from build123d import *

# Parameters (mm, degrees)
SKETCH1_W                = 15
SKETCH1_H                = 15
BOSS_EXTRUDE1_DEPTH      = 730
SKETCH2_R                = 5
BOSS_EXTRUDE2_DEPTH      = 8
SKETCH4_W                = 15
SKETCH4_H                = 15
BOSS_EXTRUDE3_DEPTH      = 198
SKETCH5_W                = 15
SKETCH5_H                = 730
BOSS_EXTRUDE4_DEPTH      = 15
BOSS_EXTRUDE5_START      = 8
SKETCH6_R                = 5
BOSS_EXTRUDE5_DEPTH      = 8
FILLET1_R                = 6
BOSS_EXTRUDE6_DEPTH      = 20
BOSS_EXTRUDE6_DEPTH_BACK = 250
SKETCH7_R                = 5


with BuildPart() as part:
    # Sketch1 → Boss-Extrude1 (new body)
    with BuildSketch(Plane(origin=(0, 0, 0), x_dir=(1, 0, 0), z_dir=(0, 1, 0))):
        Rectangle(SKETCH1_W, SKETCH1_H)
    extrude(amount=BOSS_EXTRUDE1_DEPTH)

    # Sketch2 → Boss-Extrude2 (add)
    with BuildSketch(Plane(origin=(0, 0, -7.5), x_dir=(-1, 0, 0), z_dir=(0, 0, -1))):
        with Locations(Location((0, 10, 0), (0, 0, 180))):
            Circle(SKETCH2_R)
    extrude(amount=BOSS_EXTRUDE2_DEPTH)

    # Sketch4 → Boss-Extrude3 (add)
    with BuildSketch(Plane.XY.offset(7.5)):
        with Locations((0, 450)):
            Rectangle(SKETCH4_W, SKETCH4_H)
    extrude(amount=BOSS_EXTRUDE3_DEPTH)

    # Sketch5 → Boss-Extrude4 (add)
    with BuildSketch(Plane.XY.offset(205.5)):
        with Locations((0, 365)):
            Rectangle(SKETCH5_W, SKETCH5_H)
    extrude(amount=BOSS_EXTRUDE4_DEPTH)

    # Sketch6 → Boss-Extrude5 (add)
    with BuildSketch(Plane.XY.offset(220.5).offset(BOSS_EXTRUDE5_START)):
        with Locations((0, 10)):
            Circle(SKETCH6_R)
    extrude(amount=-BOSS_EXTRUDE5_DEPTH)

    # Fillet1
    fillet1_edges = [part.edges().sort_by_distance(p)[0] for p in [
        (7.5, 0, 213),
        (-7.5, 0, 213),
        (-7.5, 0, 0),
        (7.5, 0, 0),
    ]]
    fillet(fillet1_edges, radius=FILLET1_R)

    # Sketch7 → Boss-Extrude6 (add, two sides: drawn at the far end of the back side and taken through both)
    with BuildSketch(Plane(origin=(0, 0, -7.5), x_dir=(-1, 0, 0), z_dir=(0, 0, -1)).offset(-BOSS_EXTRUDE6_DEPTH_BACK)):
        with Locations(Location((0, 720, 0), (0, 0, 180))):
            Circle(SKETCH7_R)
    extrude(amount=BOSS_EXTRUDE6_DEPTH + BOSS_EXTRUDE6_DEPTH_BACK)


solid = part.part
Input: part model. Units: mm. Frame: model coordinates. A direction names the side the tool comes from. Round coordinates to 2 decimals unless told otherwise and drop trailing zeros. Loops run counter-clockwise (first coordinate to the right, second up) from the corner with the lowest first, then second, coordinate; pieces in that order, holes last. Notation, with made-up numbers: (-11, -28.5) -> (21, -28.5) arc R11 cw to (21, -17.5) -> close; hole circle Ø4 at (22, 56.25). An arc over 180 degrees is marked (long way). Answer as a JSON object with one key per item and string values. Group by question number.
1) Section query A-A on z = 103. Output: boundary loops of the cut face in (x, y), plus the area to 3 significant figures.
2) Ray query, L1, parallel to Z at x = -3.75, y = 297; L2, parallel to Y at x = 1, z = 65; L3, parallel to Y at x = 0, z = 195.5. Return the intervals inside material, ascending.
3) Reachability of faces 1 (the flat face through (0, 224, 205.5)), 2 (the flat face through (0, 457.5, 105)), 3 (the flat face through (7.5, 447, 106)) from +Z, -Z, +X, -X, +Y, -Y: full face, straight path, thin tool, end or side. Return the list, or none.
4) Section query B-B on y = 640. Output: boundary loops of the cut face in (x, z), plus the area to 3 significant figures.
5) Draft query along Y for faces 4 (the flat face through (0, 730, 213)), 5 (the flat face through (0, 442.5, 105)), 6 (the flat face through (0, 596, 205.5)). Return one class per face: +Y half, -Y half, draft (parallel to the pull), parting line (faces both ways), or undercut.
6) Pin query (flat end, axial travel): pin 1 (1.5 mm diameter, centred on x = -2.5, z = 65.5, fed in from -Y); pin 2 (6 mm diameter, centred on x = -4.5, y = 644.5, fed in from +Z); pin 3 (3 mm diameter, centred on x = 1, y = 10, fed in from -Z). Return the tip coordinate at first contact, or that it passes through.
Reply:
{
 "1": {"outline": "(-7.5, 442.5) -> (7.5, 442.5) -> (7.5, 457.5) -> (-7.5, 457.5) -> close; circle Ø10 at (0, 720)", "area": "304 mm2"},
 "2": {"L1": "z = -7.5 to 7.5, 205.5 to 220.5", "L2": "y = 442.5 to 457.5, 715.1 to 724.9", "L3": "y = 442.5 to 457.5, 715 to 725"},
 "3": {"face 1": "+X, -X, -Y", "face 2": "+X, -X", "face 3": "+Z, -Z, +X, +Y, -Y"},
 "4": {"outline": "(-7.5, -7.5) -> (7.5, -7.5) -> (7.5, 7.5) -> (-7.5, 7.5) -> close; (-7.5, 205.5) -> (7.5, 205.5) -> (7.5, 220.5) -> (-7.5, 220.5) -> close", "area": "450 mm2"},
 "5": {"face 4": "+Y half", "face 5": "-Y half", "face 6": "undercut"},
 "6": {"pin 1": "stops at y = 442.5", "pin 2": "stops at z = 220.5", "pin 3": "stops at z = -15.5"}
}
